from build123d import *

# Parameters (mm, degrees)
BOSS_EXTRUDE1_DEPTH = 30
SKETCH2_R           = 14
BOSS_EXTRUDE2_DEPTH = 10
SKETCH3_R           = 9
BOSS_EXTRUDE3_DEPTH = 15
BOSS_EXTRUDE4_START = 10
SKETCH4_R           = 14
BOSS_EXTRUDE4_DEPTH = 10
BOSS_EXTRUDE5_START = 15
SKETCH5_R           = 9
BOSS_EXTRUDE5_DEPTH = 15
SKETCH6_R           = 9
BOSS_EXTRUDE6_DEPTH = 20
CUT_EXTRUDE1_START  = -8
SKETCH7_R           = 10.265478639
SKETCH7_R_2         = 7.147971295
CUT_EXTRUDE1_DEPTH  = 3
CHAMFER1_SIZE       = 2
SKETCH8_R           = 2.5
CUT_EXTRUDE2_DEPTH  = 6


with BuildPart() as part:
    # Sketch1 → Boss-Extrude1 (new body)
    with BuildSketch(Plane.XY):
        Polygon((0, 0), (0, 30), (-25, 30), (-25, 60), (55, 60), (55, 30), (30, 30), (30, 0), align=None)
    extrude(amount=BOSS_EXTRUDE1_DEPTH)

    # Sketch2 → Boss-Extrude2 (add)
    with BuildSketch(Plane(origin=(55, 0, 0), x_dir=(0, 0, -1), z_dir=(1, 0, 0))):
        with Locations(Location((-15, 45, 0), (0, 0, 270))):
            Circle(SKETCH2_R)
    extrude(amount=BOSS_EXTRUDE2_DEPTH)

    # Sketch3 → Boss-Extrude3 (add)
    with BuildSketch(Plane(origin=(65, 0, 0), x_dir=(0, 0, -1), z_dir=(1, 0, 0))):
        with Locations((-15, 45)):
            Circle(SKETCH3_R)
    extrude(amount=BOSS_EXTRUDE3_DEPTH)

    # Sketch4 → Boss-Extrude4 (add)
    with BuildSketch(Plane.ZY.offset(25).offset(BOSS_EXTRUDE4_START)):
        with Locations(Location((15, 45, 0), (0, 0, 270))):
            Circle(SKETCH4_R)
    extrude(amount=-BOSS_EXTRUDE4_DEPTH)

    # Sketch5 → Boss-Extrude5 (add)
    with BuildSketch(Plane.ZY.offset(35).offset(BOSS_EXTRUDE5_START)):
        with Locations(Location((15, 45, 0), (0, 0, 180))):
            Circle(SKETCH5_R)
    extrude(amount=-BOSS_EXTRUDE5_DEPTH)

    # Sketch6 → Boss-Extrude6 (add)
    with BuildSketch(Plane(origin=(0, 0, 0), x_dir=(-1, 0, 0), z_dir=(0, -1, 0))):
        with Locations((-15, -15)):
            Circle(SKETCH6_R)
    extrude(amount=BOSS_EXTRUDE6_DEPTH)

    # Sketch7 → Cut-Extrude1 (cut)
    with BuildSketch(Plane(origin=(0, -20, 0), x_dir=(-1, 0, 0), z_dir=(0, -1, 0)).offset(CUT_EXTRUDE1_START)):
        with Locations((-15, -15)):
            Circle(SKETCH7_R)
        with Locations(Location((-15, -15, 0), (0, 0, 180))):
            Circle(SKETCH7_R_2, mode=Mode.SUBTRACT)
    extrude(amount=-CUT_EXTRUDE1_DEPTH, mode=Mode.SUBTRACT)

    # Chamfer1
    chamfer1_edges = [part.edges().sort_by_distance(p)[0] for p in [
        (24, -20, 15),
    ]]
    chamfer(chamfer1_edges, length=CHAMFER1_SIZE)

    # Sketch8 → Cut-Extrude2 (cut)
    with BuildSketch(Plane(origin=(0, 0, 0), x_dir=(-1, 0, 0), z_dir=(0, 0, -1))):
        with Locations((-50, 45)):
            Circle(SKETCH8_R)
        with Locations((20, 45)):
            Circle(SKETCH8_R)
    extrude(amount=-CUT_EXTRUDE2_DEPTH, mode=Mode.SUBTRACT)


solid = part.part
Read the model definition and answer for the solid it produces. Units are mm, in the model's axes. A direction names the side the tool comes from. Give positions to 0.01 mm unless a question says otherwise; leave off trailing zeros. Write each loop counter-clockwise with the first axis right and the second up, starting at its lowest first coordinate (ties: lowest second). Pieces come first, ordered by that corner, then holes. Notation, with made-up numbers: (-5.75, 23) - (26.25, 23) arc R30 ccw to (26.25, 50) - close; hole circle Ø8 at (52.25, 64). An arc over 180 degrees is marked (long way). Answer in a Markdown table with one row per item. Add a question column.
Item 1: A tool of negligible diameter and unlimited length cuts with its end or side. For faces 1 (the face through (-12, 30, 15)), 2 (the face through (47.69, 44.04, 2.96)), 3 (the face through (6.686, -14.958, 18.447)), from which of +Z, -Z, +X, -X, +Y, -Y can it reach the whole face along a straight path? Write none if from no direction.
Item 2: Find the intervals of material crossed by L1, parallel to Y at x = -20, z = 1.6; L2, parallel to X at y = 24, z = 10; L3, parallel to Y at x = -10, z = 14, in increasing order.
Item 3: Section B-B, the plane x = 15 is taken. Write down the section's boundary in (y, z).
Item 4: Determine the mould class of faces 4 (the face through (72.4, 52.59, 10.16)), 5 (the face through (15, -20, 15)), 6 (the face through (50, 45, 6)), 7 (the face through (55, 54, 4)) for opening direction Y: pulls with the +Y half, pulls with the -Y half, needs draft (parallel to the pull), parting line crosses it, or undercut.
Item 5: Flat-ended cylindrical pins translate along their axes: P1, Ø1, axis at y = 41.5, z = 3, coming from the +X side; P2, Ø6, axis at y = -1, z = 19, coming from the +X side; P3, Ø12.5, axis at x = -17.5, z = 12.5, coming from the -Y side. Find the tip coordinate at first contact, or state that the pin passes through.
Item 6: Section C-C, the plane z = 26.5 is taken. Write down the section's boundary in (x, y).
Item 7: Section A-A, the plane y = 45 is taken. Write down the section's boundary in (x, z), and give its area (3 significant figures).
Item 8: Section D-D, the plane x = 50 is taken. Write down the section's boundary in (y, z).
Recorded:
| question | item | result |
|---|---|---|
| 1 | face 1 | +Z, -Z, -X, -Y |
| 1 | face 2 | -Z |
| 1 | face 3 | -Y |
| 2 | L1 | y = 30 to 42.5, 47.5 to 60 |
| 2 | L2 | x = 0 to 30 |
| 2 | L3 | y = 30 to 60 |
| 3 | outline | (-20, 8) - (-18, 6) - (-12, 6) - (-12, 7.85) - (-9, 7.85) - (-9, 6) - (0, 6) - (0, 0) - (60, 0) - (60, 30) - (0, 30) - (0, 24) - (-9, 24) - (-9, 22.15) - (-12, 22.15) - (-12, 24) - (-18, 24) - (-20, 22) - close |
| 4 | face 4 | parting line crosses it |
| 4 | face 5 | pulls with the -Y half |
| 4 | face 6 | undercut |
| 4 | face 7 | needs draft |
| 5 | P1 | stops at x = 65 |
| 5 | P2 | stops at x = 30 |
| 5 | P3 | stops at y = 30 |
| 6 | outline | (-35, 37.02) - (-25, 37.02) - (-25, 30) - (0, 30) - (0, 0) - (30, 0) - (30, 30) - (55, 30) - (55, 37.02) - (65, 37.02) - (65, 52.98) - (55, 52.98) - (55, 60) - (-25, 60) - (-25, 52.98) - (-35, 52.98) - close |
| 7 | outline | (-50, 6) - (-35, 6) - (-35, 1) - (-25, 1) - (-25, 0) - (-22.5, 0) - (-22.5, 6) - (-17.5, 6) - (-17.5, 0) - (47.5, 0) - (47.5, 6) - (52.5, 6) - (52.5, 0) - (55, 0) - (55, 1) - (65, 1) - (65, 6) - (80, 6) - (80, 24) - (65, 24) - (65, 29) - (55, 29) - (55, 30) - (-25, 30) - (-25, 29) - (-35, 29) - (-35, 24) - (-50, 24) - close |
| 7 | area | 3,440 mm2 |
| 8 | outline | (30, 0) - (42.5, 0) - (42.5, 6) - (47.5, 6) - (47.5, 0) - (60, 0) - (60, 30) - (30, 30) - close |
